```python
from build123d import *

# Parameters (mm, degrees)
SKETCH_1_W             = 86
SKETCH_1_H             = 60
EXTRUDE_1_DEPTH        = 46
SKETCH_2_W             = 74
SKETCH_2_H             = 48
CUT_EXTRUDE_1_DEPTH    = 41
FILLET_1_R             = 5
SKETCH_3_R             = 7
CUT_EXTRUDE_3_DEPTH    = 7
CUT_EXTRUDE_START      = -7
SKETCH_4_R             = 7
SKETCH_4_R_2           = 2.25
CUT_EXTRUDE_4_DEPTH    = 7
SKETCH_5_R             = 8.5
CUT_EXTRUDE_5_DEPTH    = 7
HOLE_WIZARD_M3_2_D     = 2.5
HOLE_WIZARD_M3_2_DEPTH = 8.5
HOLE_WIZARD_M3_2_TIP   = 0.751075774
HOLE_WIZARD_M3_3_D     = 2.5
HOLE_WIZARD_M3_3_DEPTH = 8.5
HOLE_WIZARD_M3_3_TIP   = 0.751075774
FILLET_2_R             = 2


with BuildPart() as part:
    # 草图1 → 凸台-拉伸1 (new body)
    with BuildSketch(Plane.XY):
        Rectangle(SKETCH_1_W, SKETCH_1_H)
    extrude(amount=EXTRUDE_1_DEPTH)

    # 草图2 → 切除-拉伸1 (cut)
    with BuildSketch(Plane(origin=(0, 0, 0), x_dir=(-1, 0, 0), z_dir=(0, 0, -1))):
        Rectangle(SKETCH_2_W, SKETCH_2_H)
    extrude(amount=-CUT_EXTRUDE_1_DEPTH, mode=Mode.SUBTRACT)

    # 圆角1
    fillet_1_edges = [part.edges().sort_by_distance(p)[0] for p in [
        (-37, -24, 20.5),
        (37, -24, 20.5),
        (37, 24, 20.5),
        (-37, 24, 20.5),
    ]]
    fillet(fillet_1_edges, radius=FILLET_1_R)

    # 草图3 → 切除-拉伸3 (cut)
    with BuildSketch(Plane.XZ.offset(30)):
        with Locations(Location((-5, 16, 0), (0, 0, 270))):
            Circle(SKETCH_3_R)
        with BuildLine():
            Line((25, 11.75), (29, 11.75))
            ThreePointArc((29, 11.75), (31.75, 9), (29, 6.25))
            Line((29, 6.25), (25, 6.25))
            ThreePointArc((25, 6.25), (22.25, 9), (25, 11.75))
        make_face()
        with BuildLine():
            Line((25, 33.75), (29, 33.75))
            ThreePointArc((29, 33.75), (31.75, 31), (29, 28.25))
            Line((29, 28.25), (25, 28.25))
            ThreePointArc((25, 28.25), (22.25, 31), (25, 33.75))
        make_face()
        with BuildLine():
            Line((-29, 33.75), (-25, 33.75))
            ThreePointArc((-25, 33.75), (-22.25, 31), (-25, 28.25))
            Line((-25, 28.25), (-29, 28.25))
            ThreePointArc((-29, 28.25), (-31.75, 31), (-29, 33.75))
        make_face()
        with BuildLine():
            Line((-29, 11.75), (-25, 11.75))
            ThreePointArc((-25, 11.75), (-22.25, 9), (-25, 6.25))
            Line((-25, 6.25), (-29, 6.25))
            ThreePointArc((-29, 6.25), (-31.75, 9), (-29, 11.75))
        make_face()
    extrude(amount=-CUT_EXTRUDE_3_DEPTH, mode=Mode.SUBTRACT)

    # 草图4 → 切除-拉伸4 (cut)
    with BuildSketch(Plane(origin=(0, 30, 0), x_dir=(1, 0, 0), z_dir=(0, 1, 0)).offset(CUT_EXTRUDE_START)):
        with Locations(Location((-5, -16, 0), (0, 0, 90))):
            Circle(SKETCH_4_R)
        with Locations(Location((13.186533479, -5.5, 0), (0, 0, 270))):
            Circle(SKETCH_4_R_2)
        with Locations(Location((-5, -37, 0), (0, 0, 270))):
            Circle(SKETCH_4_R_2)
        with Locations(Location((-23.186533479, -5.5, 0), (0, 0, 270))):
            Circle(SKETCH_4_R_2)
    extrude(amount=CUT_EXTRUDE_4_DEPTH, mode=Mode.SUBTRACT)

    # 草图5 → 切除-拉伸5 (cut)
    with BuildSketch(Plane.ZY.offset(43)):
        with Locations(Location((16, 0, 0), (0, 0, 270))):
            Circle(SKETCH_5_R)
    extrude(amount=-CUT_EXTRUDE_5_DEPTH, mode=Mode.SUBTRACT)

    # M3 螺纹孔2
    with Locations(Plane(origin=(-43, 0, 29.5), x_dir=(0, -1, 0), z_dir=(-1, 0, 0))):
        with Locations((0, 0), (11.691342951, -20.25), (-11.691342951, -20.25)):
            Hole(HOLE_WIZARD_M3_2_D / 2, depth=HOLE_WIZARD_M3_2_DEPTH)
            with Locations((0, 0, -(HOLE_WIZARD_M3_2_DEPTH + HOLE_WIZARD_M3_2_TIP / 2))):  # 118° drill point
                Cone(0, HOLE_WIZARD_M3_2_D / 2, HOLE_WIZARD_M3_2_TIP, mode=Mode.SUBTRACT)

    # M3 螺纹孔3
    with Locations(Plane(origin=(39.5, 25, 0), x_dir=(-1, 0, 0), z_dir=(0, 0, -1))):
        with Locations((0, 0), (79, 0), (79, -50), (0, -50)):
            Hole(HOLE_WIZARD_M3_3_D / 2, depth=HOLE_WIZARD_M3_3_DEPTH)
            with Locations((0, 0, -(HOLE_WIZARD_M3_3_DEPTH + HOLE_WIZARD_M3_3_TIP / 2))):  # 118° drill point
                Cone(0, HOLE_WIZARD_M3_3_D / 2, HOLE_WIZARD_M3_3_TIP, mode=Mode.SUBTRACT)

    # 圆角2
    fillet_2_edges = [part.edges().sort_by_distance(p)[0] for p in [
        (-43, 0, 46),
        (0, -30, 46),
        (43, 0, 46),
        (0, 30, 46),
        (43, -30, 23),
        (-43, -30, 23),
        (-43, 30, 23),
        (43, 30, 23),
    ]]
    fillet(fillet_2_edges, radius=FILLET_2_R)


solid = part.part
```
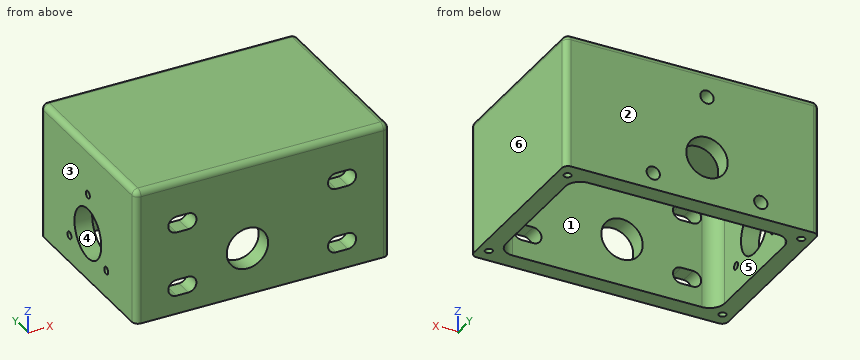
For this review, take the finished solid that the model builds, in its own axes (mm). Face numbers are marked on the shaded views. A direction names the side the tool comes from. Give positions to 0.01 mm unless a question says otherwise; leave off trailing zeros. Loops run counter-clockwise (first coordinate to the right, second up) from the corner with the lowest first, then second, coordinate; pieces in that order, holes last. Notation, with made-up numbers: M 63,-26.75 L 110,-26.75 A26 ccw 110,3.25 Z; hole C 59,1.5 d8. An arc over 180 degrees is marked long. One line per item, written item: value. Start each with the question number.
Q1. Machinability: for the marked faces 4, 5 and 6, which of the approach directions +Z, -Z, +X, -X, +Y, -Y give a long, thin tool a straight path to every point of the face, cutting with its end or side? Answer none if there is none.
Q2. Add section D-D (y = -16). Give the boundary of the cut face in (x, z).
Q3. Draft analysis for pull direction Y (two halves, no side actions). For the marked faces 1, 2 and 3, state which applies: released by +Y, released by -Y, zero draft, split by the parting line, or undercut.
Q4. For L1, parallel to X at y = -25, z = 4; L2, parallel to X at y = -13.5, z = 37; L3, parallel to Y at x = -0.5, z = 31, list the stretches that pass through material, from the lowest coordinate up.
Q5. Add section A-A (y = 4). Give the boundary of the cut face in (x, z).
Q6. Add section B-B (z = 16). Give the boundary of the cut face in (x, y).
Q7. Clearance check with flat-ended pins moving along their axes: pin 1 Ø6 at (x, y) = (2.5, -15.5) entering from -Z; pin 2 Ø2 at (x, y) = (-39.5, 25) entering from -Z; pin 3 Ø2 at (y, z) = (-3.5, 10.5) entering from -X. State where each tip first meets the part, or that it passes through.
Q8. Add section C-C (x = 30). Give the boundary of the cut face in (y, z), and give its area (3 significant figures).
Reply:
1. face 4: -X
1. face 5: -Z
1. face 6: +Z, -Z, +X, +Y, -Y
2. outline: M -43,0 L -37,0 L -37,41 L 37,41 L 37,0 L 43,0 L 43,44 A2 ccw 41,46 L -41,46 A2 ccw -43,44 Z
3. face 1: undercut
3. face 2: released by +Y
3. face 3: zero draft
4. L1: -43 to -40.75, -38.25 to 38.25, 40.75 to 43
4. L2: -43 to -37, 37 to 43
4. L3: -30 to -24, 24 to 30
5. outline: M -43,0 L -37,0 L -37,8.5 L -43,8.5 Z; M -43,23.5 L -37,23.5 L -37,41 L 37,41 L 37,0 L 43,0 L 43,44 A2 ccw 41,46 L -41,46 A2 ccw -43,44 Z
6. outline: M -43,-28 A2 ccw -41,-30 L -12,-30 L -12,-24 L -32,-24 A5 cw -37,-19 L -37,-8.5 L -43,-8.5 Z; M -43,8.5 L -37,8.5 L -37,19 A5 cw -32,24 L -12,24 L -12,30 L -41,30 A2 ccw -43,28 Z; M 2,-30 L 41,-30 A2 ccw 43,-28 L 43,28 A2 ccw 41,30 L 2,30 L 2,24 L 32,24 A5 cw 37,19 L 37,-19 A5 cw 32,-24 L 2,-24 Z
7. pin 1: z = 41
7. pin 2: z = 8.65
7. pin 3: x = 37
8. outline: M -30,0 L -24,0 L -24,6.44 L -30,6.44 Z; M -30,11.56 L -24,11.56 L -24,28.44 L -30,28.44 Z; M -30,33.56 L -24,33.56 L -24,41 L 24,41 L 24,0 L 30,0 L 30,44 A2 ccw 28,46 L -28,46 A2 ccw -30,44 Z
8. area: 729 mm²
